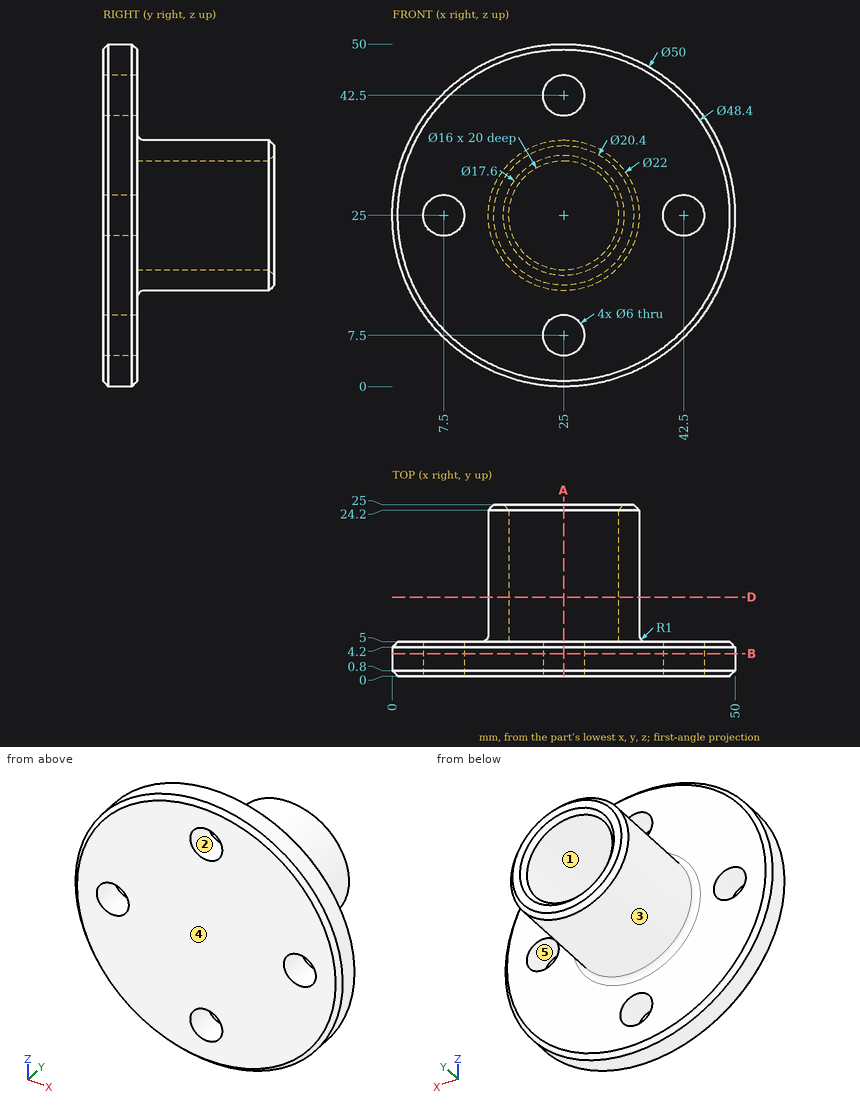
Input: dimensioned drawing with shaded views. Units: mm. Origin: part minimum x, y, z. A direction names the side the tool comes from. Round coordinates to 2 decimals unless told otherwise and drop trailing zeros. Write each loop counter-clockwise with the first axis right and the second up, starting at its lowest first coordinate (ties: lowest second). Pieces come first, ordered by that corner, then holes. Notation, with made-up numbers: (39, -1) - (83, -1) arc R32 ccw to (83, 28) - close; hole circle Ø6 at (-23.5, 60). An arc over 180 degrees is marked (long way). Write item = value, one per line.
(1) Pull-direction query (Z, two-part tool) for the marked faces 3, 4 and 5; classes: +Z half, -Z half, draft (parallel to the pull), parting line (faces both ways), or undercut.
Geometry check:
face_3 = parting line
face_4 = draft
face_5 = undercut
(2) Section query A-A on x = 25. State how many separate pieces and enclosed holes the cut face has, then the cut area to 3 significant figures.
Geometry check:
separate_pieces = 3
enclosed_holes = 0
area = 308 mm^2
(3) Access query for the marked faces 1 and 2. Directions: +Z, -Z, +X, -X, +Y, -Y. A direction counts if a zero-diameter tool reaches every point of the face in a straight line with its end or side. Return the directions, or none.
Geometry check:
face_1 = +Y
face_2 = +Y, -Y
(4) Section query D-D on y = 11.5. Output: boundary loops of the cut face in (x, z), then the cut area to 3 significant figures.
Geometry check:
outline = circle Ø22 at (25, 25); hole circle Ø16 at (25, 25)
area = 179 mm^2
(5) Material intervals for probe 1 along X at (y, z) = (1.55, 25); probe 2 along Z at (x, y) = (22.5, 4.5); probe 3 along Z at (x, y) = (25.5, 20), sorted ascending.
Geometry check:
probe_1 = 0 to 4.5, 10.5 to 39.5, 45.5 to 50
probe_2 = 0.43 to 5.84, 9.16 to 40.84, 44.16 to 49.57
probe_3 = 14.01 to 17.02, 32.98 to 35.99
(6) Contact query for flat-ended pins moving along their axis: pin 1 Ø4 at (x, z) = (8, 39) entering from +Y; pin 2 Ø8 at (y, z) = (6.5, 7) entering from -X; pin 3 Ø6 at (x, y) = (29.5, 5) entering from +Z. Output: stop coordinate, or through.
Geometry check:
pin_1 = 5
pin_2 = 4.8
pin_3 = 49.95
(7) Section query B-B on y = 3.25. Output: boundary loops of the cut face in (x, z), then the cut area to 3 significant figures.
Geometry check:
outline = circle Ø50 at (25, 25); hole circle Ø6 at (7.5, 25); hole circle Ø6 at (25, 7.5); hole circle Ø6 at (25, 42.5); hole circle Ø6 at (42.5, 25)
area = 1,850 mm^2
